from build123d import *

# Parameters (mm, degrees)
SKETCH_1_R           = 20
BOSS_EXTRUDE_1_DEPTH = 60
SKETCH_2_R           = 16.5
BOSS_EXTRUDE_2_DEPTH = 40


with BuildPart() as part:
    # Sketch 1 → Boss-Extrude 1 (new, symmetric)
    with BuildSketch(Plane.XY):
        Circle(SKETCH_1_R)
    extrude(amount=BOSS_EXTRUDE_1_DEPTH, both=True)

    # Sketch 2 → Boss-Extrude 2 (add)
    with BuildSketch(Plane.XY.offset(60)):
        Circle(SKETCH_2_R)
    boss_extrude_2 = extrude(amount=BOSS_EXTRUDE_2_DEPTH)

    # Mirror 1: Boss-Extrude 2 across plane
    add(boss_extrude_2.mirror(Plane.XY))


solid = part.part
Source: CAD feature listing. Evaluate the final solid. Frame: model axes, mm. A direction names the side the tool comes from. Coordinates: 2 decimals unless noted, no trailing zeros. Write each loop counter-clockwise with the first axis right and the second up, starting at its lowest first coordinate (ties: lowest second). Pieces come first, ordered by that corner, then holes. Notation, with made-up numbers: M 30.25,-37 L 86.25,-37 A23 cw 86.25,-3 Z; hole C 40,61.5 d11. An arc over 180 degrees is marked long. Use a Markdown table: item, result.
1) Reachability of faces 1 (the flat face through (2.9, 16.4, 60)), 2 (the flat face through (0, 0, 100)), 3 (the flat face through (2.9, 16.4, -60)) from +Z, -Z, +X, -X, +Y, -Y: full face, straight path, thin tool, end or side. Return the list, or none.
Conclusion:
| item | result |
|---|---|
| face 1 | +Z |
| face 2 | +Z, +X, -X, +Y, -Y |
| face 3 | -Z |
2) Section A-A, the plane y = 0. Output: boundary loops of the cut face in (x, z), then the cut area to 3 significant figures.
Conclusion:
| item | result |
|---|---|
| outline | M -20,-60 L -16.5,-60 L -16.5,-100 L 16.5,-100 L 16.5,-60 L 20,-60 L 20,60 L 16.5,60 L 16.5,100 L -16.5,100 L -16.5,60 L -20,60 Z |
| area | 7,440 mm^2 |
3) First-contact query: pin 1 Ø3 at (x, z) = (7.5, 39) entering from +Y; pin 2 Ø8 at (x, z) = (-5, -48) entering from -Y (3 decimals); pin 3 Ø10 at (x, z) = (-9, 25) entering from -Y. Flat tips, straight axial feed; report the tip coordinate or a pass-through.
Conclusion:
| item | result |
|---|---|
| pin 1 | stops at y = 19.08 |
| pin 2 | stops at y = -19.975 |
| pin 3 | stops at y = -19.6 |
4) Ray query, L1, parallel to Z at x = -4.5, y = -17.5; L2, parallel to Y at x = 0.5, z = -32; L3, parallel to Y at x = 5, z = 8. Return the intervals inside material, ascending.
Conclusion:
| item | result |
|---|---|
| L1 | z = -60 to 60 |
| L2 | y = -19.99 to 19.99 |
| L3 | y = -19.36 to 19.36 |
5) Section C-C, the plane z = -25. Output: boundary loops of the cut face in (x, y), then the cut area to 3 significant figures.
Conclusion:
| item | result |
|---|---|
| outline | C 0,0 d40 |
| area | 1,260 mm^2 |
